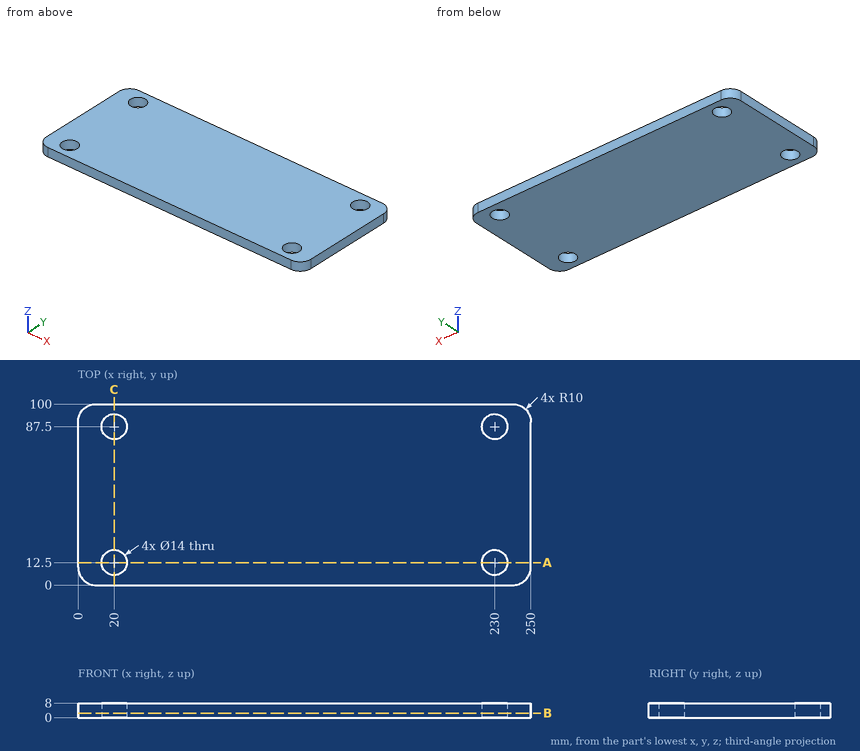
Geometry: see drawing. Coordinates: mm, zero at the bounding-box minimum. Coordinates: 2 decimals unless noted, no trailing zeros. Loops run counter-clockwise (first coordinate to the right, second up) from the corner with the lowest first, then second, coordinate; pieces in that order, holes last.
(1) Section C-C on x = 20. Return the cut outline in (y, z), then the cut area to 3 significant figures.
(2) Material intervals for probe 1 along Y at (x, z) = (230, 2.5); probe 2 along X at (y, z) = (16, 5.5); probe 3 along Y at (x, z) = (21.5, 6), sorted ascending.
(3) Section B-B on z = 2.5. Return the cut outline in (x, y).
(4) Section A-A on y = 12.5. Return the cut outline in (x, z).
Data:
1. outline: (0, 0) - (5.5, 0) - (5.5, 8) - (0, 8) - close; (19.5, 0) - (80.5, 0) - (80.5, 8) - (19.5, 8) - close; (94.5, 0) - (100, 0) - (100, 8) - (94.5, 8) - close
1. area: 576 mm2
2. probe 1: y = 0 to 5.5, 19.5 to 80.5, 94.5 to 100
2. probe 2: x = 0 to 13.94, 26.06 to 223.94, 236.06 to 250
2. probe 3: y = 0 to 5.66, 19.34 to 80.66, 94.34 to 100
3. outline: (0, 10) arc R10 ccw to (10, 0) - (240, 0) arc R10 ccw to (250, 10) - (250, 90) arc R10 ccw to (240, 100) - (10, 100) arc R10 ccw to (0, 90) - close; hole circle Ø14 at (20, 12.5); hole circle Ø14 at (20, 87.5); hole circle Ø14 at (230, 12.5); hole circle Ø14 at (230, 87.5)
4. outline: (0, 0) - (13, 0) - (13, 8) - (0, 8) - close; (27, 0) - (223, 0) - (223, 8) - (27, 8) - close; (237, 0) - (250, 0) - (250, 8) - (237, 8) - close
